The model under review builds one solid part; all positions refer to its coordinate system, in mm. A direction names the side the tool comes from. Give positions to 0.01 mm unless a question says otherwise; leave off trailing zeros. Write each loop counter-clockwise with the first axis right and the second up, starting at its lowest first coordinate (ties: lowest second). Pieces come first, ordered by that corner, then holes. Notation, with made-up numbers: M 65.25,76 L 87.25,76 A32 cw 87.25,112 Z; hole C -24,1.5 d11. An arc over 180 degrees is marked long. Write item = value, one per line. Start each with the question number.
```python
from build123d import *

# Parameters (mm, degrees)
SKETCH_6_W             = 25
SKETCH_6_H             = 20
SKETCH_6_R             = 5
EXTRUDE_4_DEPTH        = 10
SKETCH_7_R             = 5
EXTRUDE_5_DEPTH        = 367
HOLE_WIZARD_M4_1_D     = 3.3
HOLE_WIZARD_M4_1_DEPTH = 5
HOLE_WIZARD_M4_1_TIP   = 0.991420021
EXTRUDE_6_DEPTH        = 10
SKETCH_11_R            = 5
EXTRUDE_7_DEPTH        = 25
SKETCH_12_R            = 8
EXTRUDE_8_DEPTH        = 40


with BuildPart() as part:
    # 草图6 → 凸台-拉伸4 (new body)
    with BuildSketch(Plane.XY):
        with Locations((12.5, 10)):
            Rectangle(SKETCH_6_W, SKETCH_6_H)
        with Locations((10, 10)):
            Circle(SKETCH_6_R, mode=Mode.SUBTRACT)
    extrude(amount=EXTRUDE_4_DEPTH)

    # 草图7 → 凸台-拉伸5 (add)
    with BuildSketch(Plane.ZY):
        with Locations((5, 10)):
            Circle(SKETCH_7_R)
    extrude(amount=EXTRUDE_5_DEPTH)

    # M4 螺纹孔1
    with Locations(Plane(origin=(25, 0, 0), x_dir=(0, 0, -1), z_dir=(1, 0, 0))):
        with Locations((-5, 10)):
            Hole(HOLE_WIZARD_M4_1_D / 2, depth=HOLE_WIZARD_M4_1_DEPTH)
            with Locations((0, 0, -(HOLE_WIZARD_M4_1_DEPTH + HOLE_WIZARD_M4_1_TIP / 2))):  # 118° drill point
                Cone(0, HOLE_WIZARD_M4_1_D / 2, HOLE_WIZARD_M4_1_TIP, mode=Mode.SUBTRACT)

    # 草图10 → 凸台-拉伸6 (add)
    with BuildSketch(Plane.ZY.offset(367)):
        Polygon((0, 40), (10, 40), (10, 5), (0, 5), (0, 15), align=None)
    extrude(amount=EXTRUDE_6_DEPTH)

    # 草图11 → 凸台-拉伸7 (add)
    with BuildSketch(Plane(origin=(0, 40, 0), x_dir=(1, 0, 0), z_dir=(0, 1, 0))):
        with Locations(Location((-372, -5, 0), (0, 0, 270))):
            Circle(SKETCH_11_R)
    extrude(amount=EXTRUDE_7_DEPTH)

    # 草图12 → 凸台-拉伸8 (add)
    with BuildSketch(Plane.ZY.offset(100)):
        with BuildLine():
            Line((3.75, 17.395099729), (18.333333333, 19.860132972))
            ThreePointArc((18.333333333, 19.860132972), (30, 10), (18.333333333, 0.139867028))
            Line((18.333333333, 0.139867028), (3.75, 2.604900271))
            ThreePointArc((3.75, 2.604900271), (-2.5, 10), (3.75, 17.395099729))
        make_face()
        with Locations((20, 10)):
            Circle(SKETCH_12_R, mode=Mode.SUBTRACT)
    extrude(amount=EXTRUDE_8_DEPTH)


solid = part.part
```
Item 1: For faces 1 (the flat face through (15, 12, 0)), 2 (the cylindrical face through (-367.043, 52.325, 4.349)), 3 (the flat face through (-372, 23, 10)), 4 (the cylindrical face through (-119.7, 9.9, -2.5)), 5 (the flat face through (-119.72, 1.355, 11.144)), list the 3-axis set-ups (+Z, -Z, +X, -X, +Y, -Y) from which the entire face can be reached by the end or side of a thin tool; tool diameter is ignored.
Item 2: Clearance check with flat-ended pins moving along their axes: P1, Ø3, axis at x = -324, z = 5, coming from the -Y side; P2, Ø12, axis at x = -266.5, y = 14.5, coming from the -Z side; P3, Ø6, axis at x = 15.5, y = 12, coming from the +Z side. State where each tip first meets the part, or that it passes through.
Item 3: The part is to be moulded in two halves that separate along X. For faces 6 (the flat face through (-119.72, 18.61, 10.94)), 7 (the cylindrical face through (-120, 10, 30)), 8 (the flat face through (-377, 23, 5)), say which applies: released by +X, released by -X, zero draft, split by the parting line, or undercut.
Item 4: To check wall thickness, follow probe 1 along Y at (x, z) = (10, 3); probe 2 along Z at (x, y) = (23.5, 10); probe 3 along Z at (x, y) = (-107, 10.5). State the ranges of each line that lie inside material, in increasing order. Write a range as [from, to].
Item 5: We need section A-A, the plane x = -109.5. Write out the cut boundary in (y, z), and give its area (3 significant figures).
Item 6: We need section C-C, the plane y = 61. Write out the cut boundary in (x, z).
Item 7: We need section D-D, the plane x = -280. Write out the cut boundary in (y, z), and give its area (3 significant figures).
Item 8: We need section B-B, the plane z = 22. Write out the cut boundary in (x, y).
Worked out:
q1.face_1 = -Z, +X, +Y, -Y
q1.face_2 = +Y
q1.face_3 = +Z, -X, +Y, -Y
q1.face_4 = -Z
q1.face_5 = -Z, -X, -Y
q2.P1 = 5
q2.P2 = 0
q2.P3 = 10
q3.face_6 = undercut
q3.face_7 = zero draft
q3.face_8 = released by -X
q4.probe_1 = [0, 5], [15, 20]
q4.probe_2 = [0, 3.35], [6.65, 10]
q4.probe_3 = [-2.48, 12.02], [27.98, 29.99]
q5.outline = M 0.14,18.33 L 2.6,3.75 A7.5 ccw 17.4,3.75 L 19.86,18.33 A10 ccw long Z; hole C 10,20 d16
q5.area = 311 mm²
q6.outline = C -372,5 d10
q7.outline = C 10,5 d10
q7.area = 78.5 mm²
q8.outline = M -140,0.2 L -100,0.2 L -100,2.25 L -140,2.25 Z; M -140,17.75 L -100,17.75 L -100,19.8 L -140,19.8 Z
